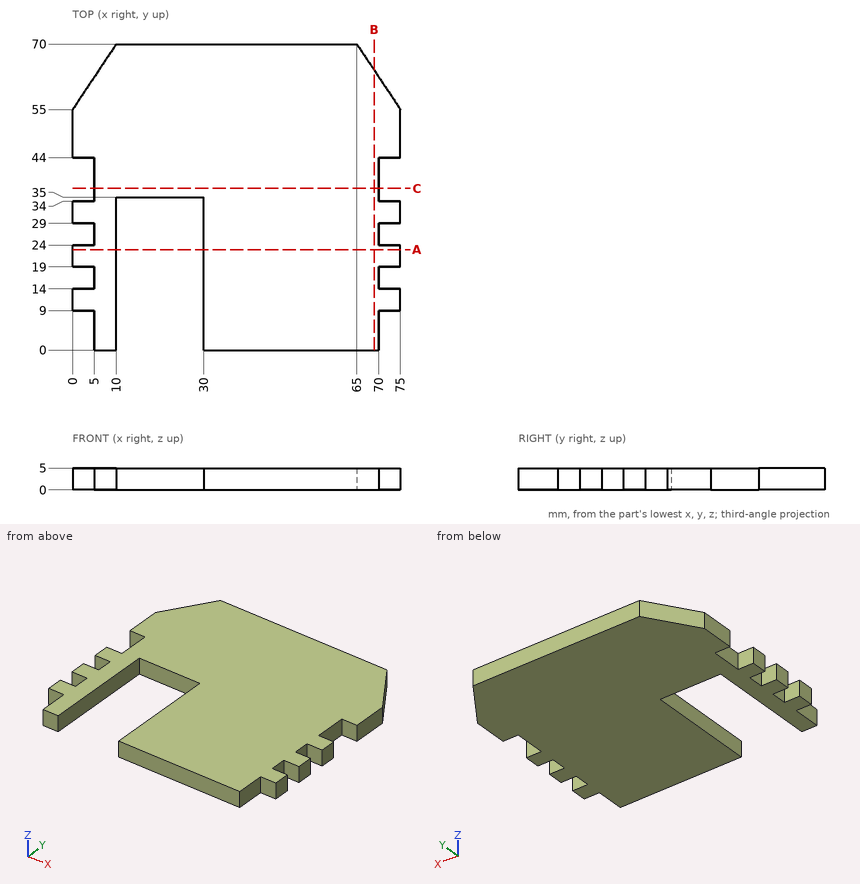
Source: three-view drawing plus pictorial views. Frame: mm from the lowest corner of the part. Coordinates: 2 decimals unless noted, no trailing zeros. Write each loop counter-clockwise with the first axis right and the second up, starting at its lowest first coordinate (ties: lowest second). Pieces come first, ordered by that corner, then holes. Notation, with made-up numbers: (24, 9.25) -> (39, 9.25) arc R23 ccw to (39, 35.25) -> close; hole circle Ø6 at (31, 47). An arc over 180 degrees is marked (long way). Write each question's results on one line, items separated by ' | '.
Item 1: Pin query (flat end, axial travel): pin 1 Ø2.5 at (x, z) = (72.5, 2) entering from +Y (3 decimals); pin 2 Ø1 at (y, z) = (7.5, 3.5) entering from +X; pin 3 Ø1.5 at (x, z) = (3.5, 1.5) entering from -Y; pin 4 Ø1 at (x, y) = (29, 21) entering from +Z. Return the tip coordinate at first contact, or that it passes through.
Conclusion:
pin 1: stops at y = 60.625 | pin 2: stops at x = 70 | pin 3: stops at y = 9 | pin 4: passes through
Item 2: Section query A-A on y = 23. Return loops of the section in (x, z), plus the area to 3 significant figures.
Conclusion:
outline: (0, 0) -> (10, 0) -> (10, 5) -> (0, 5) -> close; (30, 0) -> (75, 0) -> (75, 5) -> (30, 5) -> close | area: 275 mm^2
Item 3: Material intervals for probe 1 along X at (y, z) = (32, 0.4); probe 2 along X at (y, z) = (16, 1.5); probe 3 along Y at (x, z) = (29, 3.6), sorted ascending.
Conclusion:
probe 1: x = 0 to 10, 30 to 75 | probe 2: x = 5 to 10, 30 to 70 | probe 3: y = 35 to 70
Item 4: Section query C-C on y = 37. Return loops of the section in (x, z).
Conclusion:
outline: (5, 0) -> (70, 0) -> (70, 5) -> (5, 5) -> close
Item 5: Section query B-B on x = 69. Return loops of the section in (y, z), plus the area to 3 significant figures.
Conclusion:
outline: (0, 0) -> (64, 0) -> (64, 5) -> (0, 5) -> close | area: 320 mm^2
